Here's how the part is built. I have some questions about the finished solid (model axes, mm). A direction names the side the tool comes from. Coordinates: 2 decimals unless noted, no trailing zeros. Loops run counter-clockwise (first coordinate to the right, second up) from the corner with the lowest first, then second, coordinate; pieces in that order, holes last. Notation, with made-up numbers: (-16.75, -30.5) -> (37.25, -30.5) arc R10 cw to (37.25, -12.5) -> close; hole circle Ø6 at (84.5, 87). An arc over 180 degrees is marked (long way). Answer as a JSON object with one key per item and string values. Group by question number.
Q1. I'm going to push flat-ended pins straight in: pin 1 (10 mm diameter, centred on x = 55.5, z = -9.5, fed in from +Y); pin 2 (10 mm diameter, centred on x = 269, z = -10.5, fed in from -Y); pin 3 (4 mm diameter, centred on x = 185, z = 4, fed in from +Y). Where does each tip first touch, or does it pass through?
Q2. I need wall thicknesses on line 1 (Z direction, x = 10.5, y = 0); line 2 (Y direction, x = 186, z = 1.5); line 3 (Y direction, x = 471, z = -0.5). Which ranges of each line are inside material? Lowest first, please.
Q3. On a 3-axis mill with a long thin cutter (end or side, diameter ignored), from which of +Z, -Z, +X, -X, +Y, -Y can I reach the whole of each face in a straight line? I mean faces 1 (the flat face through (22, 0, -13.5)), 2 (the flat face through (22, 0, 13.5)), 3 (the flat face through (525, 0, 0)). Say none if no direction works.
Q4. I want a section at A-A on x = 158.5. Write out the boundary of the cut face in (y, z).
```python
from build123d import *

# Parameters (mm, degrees)
SKETCH3_W          = 54
SKETCH3_H          = 120
SKETCH3_W_2        = 27
SKETCH3_H_2        = 60
CUT_EXTRUDE1_DEPTH = 15


with BuildPart() as part:
    # Sketch1 → Revolve1 (revolve)
    with BuildSketch(Plane.XY, mode=Mode.PRIVATE) as revolve1_sk:
        Polygon((0, 0), (0, 14), (1, 15), (524, 15), (525, 14), (525, 0), align=None)
    revolve(revolve1_sk.sketch.rotate(Axis((525, 0, 0), (-1, 0, 0)), 180), axis=Axis((525, 0, 0), (-1, 0, 0)))

    # Sketch2 → Cut-Revolve1 (revolve, cut)
    with BuildSketch(Plane.XY, mode=Mode.PRIVATE) as cut_revolve1_sk:
        Polygon((0, 0), (0, 4), (0.6765, 3.3235), (17.6, 3.3235), (19.51882362, 0), align=None)
    revolve(cut_revolve1_sk.sketch.rotate(Axis((19.51882362, 0, 0), (-1, 0, 0)), 180), axis=Axis((19.51882362, 0, 0), (-1, 0, 0)), mode=Mode.SUBTRACT)

    # Sketch3 → Cut-Extrude1 (cut)
    with BuildSketch(Plane(origin=(15, 0, 0), x_dir=(0, 0, -1), z_dir=(1, 0, 0))):
        Rectangle(SKETCH3_W, SKETCH3_H)
        Rectangle(SKETCH3_W_2, SKETCH3_H_2, mode=Mode.SUBTRACT)
    extrude(amount=CUT_EXTRUDE1_DEPTH, mode=Mode.SUBTRACT)


solid = part.part
```
Result set:
{
 "1": {"pin 1": "stops at y = 14.31", "pin 2": "stops at y = -13.96", "pin 3": "stops at y = 14.87"},
 "2": {"line 1": "z = -15 to -3.32, 3.32 to 15", "line 2": "y = -14.92 to 14.92", "line 3": "y = -14.99 to 14.99"},
 "3": {"face 1": "-Z, +Y, -Y", "face 2": "+Z, +Y, -Y", "face 3": "+Z, -Z, +X, +Y, -Y"},
 "4": {"outline": "circle Ø30 at (0, 0)"}
}
